Design review of the part built by this model. Coordinates are the model's own, in mm. Face numbers are marked on the shaded views. A direction names the side the tool comes from. Coordinates: 2 decimals unless noted, no trailing zeros. Write each loop counter-clockwise with the first axis right and the second up, starting at its lowest first coordinate (ties: lowest second). Pieces come first, ordered by that corner, then holes. Notation, with made-up numbers: (-36.75, -3) -> (-20.75, -3) arc R18 ccw to (-20.75, 16) -> close; hole circle Ø4 at (20.5, 11.5). An arc over 180 degrees is marked (long way). One line per question, with ' | ' between items. Start each with the question number.
Q1. Add section B-B on z = 283.5. State the section outline as (x, y) points, and give its area (3 significant figures).
Q2. For the marked faces 1 and 2, list the 3-axis set-ups (+Z, -Z, +X, -X, +Y, -Y) from which the entire face can be reached by the end or side of a thin tool; tool diameter is ignored.
Q3. Add section A-A on y = 20. State the section outline as (x, z) points, and give its area (3 significant figures).
Q4. Draft analysis for pull direction Y (two halves, no side actions). For the marked faces 3, 4, 5 and 6, state which applies: pulls with the +Y half, pulls with the -Y half, needs draft (parallel to the pull), parting line crosses it, or undercut.
Q5. Wall thickness on probe 1 along Y at (x, z) = (17, 121): over which ranges is the line inside the solid? List them lowest first.
from build123d import *

# Parameters (mm, degrees)
SKETCH_1_W      = 50
SKETCH_1_H      = 50
SKETCH_1_W_2    = 44
SKETCH_1_H_2    = 44
EXTRUDE_2_DEPTH = 340


with BuildPart() as part:
    # 草图1 → 凸台-拉伸2 (new body)
    with BuildSketch(Plane.XY):
        with Locations((25, 25)):
            Rectangle(SKETCH_1_W, SKETCH_1_H)
        with Locations((25, 25)):
            Rectangle(SKETCH_1_W_2, SKETCH_1_H_2, mode=Mode.SUBTRACT)
    extrude(amount=EXTRUDE_2_DEPTH)


solid = part.part
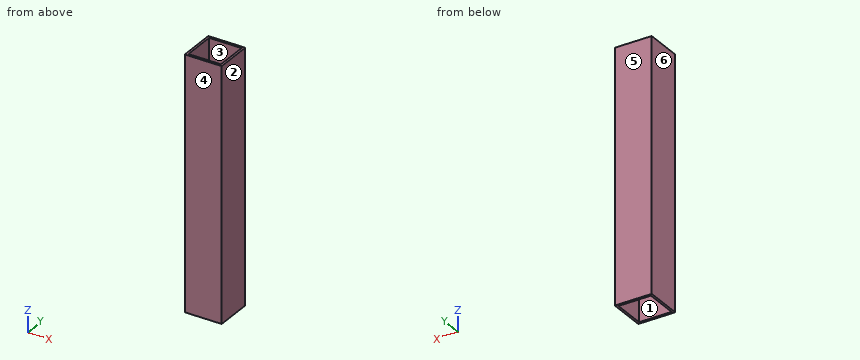
Output values:
1) outline: (0, 0) -> (50, 0) -> (50, 50) -> (0, 50) -> close; hole (3, 3) -> (47, 3) -> (47, 47) -> (3, 47) -> close | area: 564 mm2
2) face 1: +Z, -Z | face 2: +Z, -Z, +X, +Y, -Y
3) outline: (0, 0) -> (3, 0) -> (3, 340) -> (0, 340) -> close; (47, 0) -> (50, 0) -> (50, 340) -> (47, 340) -> close | area: 2,040 mm2
4) face 3: undercut | face 4: pulls with the -Y half | face 5: pulls with the +Y half | face 6: needs draft
5) probe 1: y = 0 to 3, 47 to 50
